from build123d import *

# Parameters (mm, degrees)
SKETCH_1_R       = 25
EXTRUDE_1_DEPTH  = 195
SKETCH_2_W       = 15
SKETCH_2_H       = 15
EXTRUDE_2_DEPTH  = 225
MOVE_FACE_1_BY   = 3
MOVE_FACE_1_2_BY = 3
MOVE_FACE_1_3_BY = 3
MOVE_FACE_1_4_BY = 3


with BuildPart() as part:
    # 草图1 → 凸台-拉伸1 (new, symmetric)
    with BuildSketch(Plane.XY):
        Circle(SKETCH_1_R)
    extrude(amount=EXTRUDE_1_DEPTH, both=True)

    # 草图2 → 凸台-拉伸2 (add, symmetric)
    with BuildSketch(Plane.XY):
        Rectangle(SKETCH_2_W, SKETCH_2_H)
    extrude(amount=EXTRUDE_2_DEPTH, both=True)

    # Move Face 1: a face moved outward by 3.0
    extrude(part.faces().sort_by_distance((7.5, 0, -210))[0], amount=MOVE_FACE_1_BY, dir=(1, 0, 0))

    # Move Face 1 2: a face moved outward by 3.0
    extrude(part.faces().sort_by_distance((0, -7.5, -210))[0], amount=MOVE_FACE_1_2_BY, dir=(0, -1, 0))

    # Move Face 1 3: a face moved outward by 3.0
    extrude(part.faces().sort_by_distance((-7.5, 0, -210))[0], amount=MOVE_FACE_1_3_BY, dir=(-1, 0, 0))

    # Move Face 1 4: a face moved outward by 3.0
    extrude(part.faces().sort_by_distance((0, 7.5, -210))[0], amount=MOVE_FACE_1_4_BY, dir=(0, 1, 0))


solid = part.part
For this review, take the finished solid that the model builds, in its own axes (mm). A direction names the side the tool comes from. Round coordinates to 2 decimals unless told otherwise and drop trailing zeros. Order: outer loops, then holes, each group sorted by start corner. A loop starts at its lowest first (then second) coordinate and runs counter-clockwise, first axis right, second up. Notation, with made-up numbers: (40.25, -18.75) -> (90.25, -18.75) arc R23 cw to (90.25, -1.75) -> close; hole circle Ø4 at (75.25, -33.75). An arc over 180 degrees is marked (long way). Put each result on its own line as item: value.
Q1. For probe 1 along Z at (x, y) = (-13.5, -1); probe 2 along X at (y, z) = (-2, 190), list the stretches that pass through material, from the lowest coordinate up. Write a range as [from, to].
Check result:
probe 1: [-195, 195]
probe 2: [-24.92, 24.92]
Q2. Insertion check: pin 1 Ø5 at (y, z) = (-3.5, -46) entering from +X; pin 2 Ø3 at (x, z) = (17, 93.5) entering from +Y; pin 3 Ø10 at (y, z) = (13.5, 142.5) entering from +X. Each pin has a flat end and moves straight along its axis. Give the tip position at first contact, or say it passes through.
Check result:
pin 1: x = 24.98
pin 2: y = 19.62
pin 3: x = 23.51
Q3. Machinability: for faces 1 (the flat face through (0, 10.5, -210)), 2 (the flat face through (0, 7.5, 210)), 3 (the flat face through (0, -7.5, 210)), which of the approach directions +Z, -Z, +X, -X, +Y, -Y give a long, thin tool a straight path to every point of the face, cutting with its end or side? Answer none if there is none.
Check result:
face 1: -Z, +X, -X, +Y
face 2: +Z, +X, -X, +Y
face 3: +Z, +X, -X, -Y
Q4. Add section C-C on z = 100. Write out the cut boundary in (x, y), plus the area to 3 significant figures.
Check result:
outline: circle Ø50 at (0, 0)
area: 1,960 mm2
Q5. Add section A-A on x = 0. Write out the cut boundary in (y, z), plus the area to 3 significant figures.
Check result:
outline: (-25, -195) -> (-10.5, -195) -> (-10.5, -225) -> (10.5, -225) -> (10.5, -195) -> (25, -195) -> (25, 195) -> (7.5, 195) -> (7.5, 225) -> (-7.5, 225) -> (-7.5, 195) -> (-25, 195) -> close
area: 20,600 mm2
Q6. Add section D-D on y = -21. Write out the cut boundary in (x, z).
Check result:
outline: (-13.56, -195) -> (13.56, -195) -> (13.56, 195) -> (-13.56, 195) -> close
